from build123d import *

# Parameters (mm, degrees)
SKETCH_1_W              = 95
SKETCH_1_H              = 65
EXTRUDE_1_DEPTH         = 12
HOLE_WIZARD_6_5_6_5_1_D = 6.5
CHAMFER_1_SIZE          = 5
SKETCH_4_R              = 26
CUT_EXTRUDE_1_DEPTH     = 59.792006259
HOLE_WIZARD_M5_1_D      = 4.2
CHAMFER_2_SIZE          = 1


with BuildPart() as part:
    # 草图1 → 凸台-拉伸1 (new body)
    with BuildSketch(Plane.XY):
        Rectangle(SKETCH_1_W, SKETCH_1_H)
    extrude(amount=EXTRUDE_1_DEPTH)

    # Ø6.5 (6.5) 直径孔1 (through all)
    with Locations(Plane.XY.offset(12)):
        with Locations((-40, -26.5), (40, -26.5)):
            Hole(HOLE_WIZARD_6_5_6_5_1_D / 2)

    # 倒角1
    chamfer_1_edges = [part.edges().sort_by_distance(p)[0] for p in [
        (-47.5, 32.5, 6),
        (47.5, 32.5, 6),
    ]]
    chamfer(chamfer_1_edges, length=CHAMFER_1_SIZE)

    # 草图4 → 切除-拉伸1 (cut, through all)
    with BuildSketch(Plane(origin=(0, 0, 0), x_dir=(-1, 0, 0), z_dir=(0, 0, -1))):
        with Locations((0, 2.5)):
            Circle(SKETCH_4_R)
    extrude(amount=-CUT_EXTRUDE_1_DEPTH, mode=Mode.SUBTRACT)

    # M5 螺纹孔1 (through all)
    with Locations(Plane.XY.offset(12)):
        with Locations((-24.748737342, 27.25), (24.748737342, 27.25), (24.748737342, -22.25), (-24.748737342, -22.25)):
            Hole(HOLE_WIZARD_M5_1_D / 2)

    # 倒角2
    chamfer_2_edges = [part.edges().sort_by_distance(p)[0] for p in [
        (0, -32.5, 12),
        (0, 32.5, 0),
        (0, 32.5, 12),
        (-47.5, -2.5, 0),
        (-45, 30, 0),
        (45, 30, 0),
        (-47.5, -2.5, 12),
        (-45, 30, 12),
        (45, 30, 12),
        (47.5, -2.5, 12),
        (0, -32.5, 0),
        (47.5, -2.5, 0),
        (47.5, -32.5, 6),
        (-47.5, -32.5, 6),
    ]]
    chamfer(chamfer_2_edges, length=CHAMFER_2_SIZE)


solid = part.part
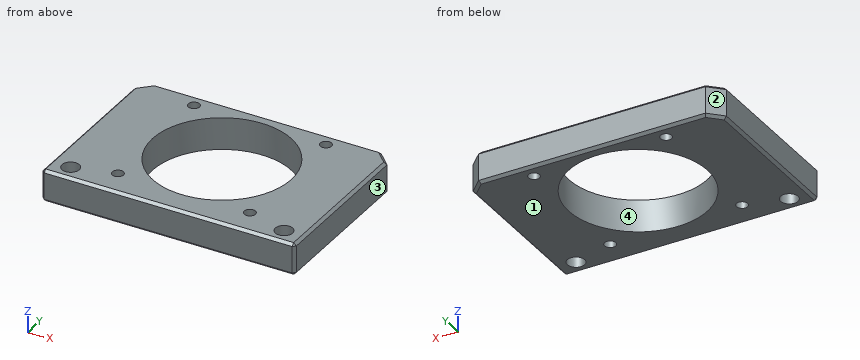
Could you check a few things on this model? Use its own coordinates, in mm. Face numbers are marked on the shaded views. Coordinates: 2 decimals unless noted, no trailing zeros. Order: outer loops, then holes, each group sorted by start corner. A loop starts at its lowest first (then second) coordinate and runs counter-clockwise, first axis right, second up.
Q1. Thinking about a two-plate mould opening in X: for the marked faces 1, 2, 3 and 4, which applies, released by +X, released by -X, zero draft, split by the parting line, or undercut?
Q2. Suppose I cut it at D-D on z = 3. Please give me the cut outline in (x, y), and give its area (3 significant figures).
Q3. Suppose I cut it at C-C on y = 2.5. Please give me the cut outline in (x, z), and give its area (3 significant figures).
Q4. Please list where these lines run through material, in increasing order: L1, parallel to Y at x = 40, z = 5; L2, parallel to X at y = 26.5, z = 2; L3, parallel to Y at x = -4, z = 3.25.
Q5. Suppose I cut it at A-A on x = -40. Please give me the cut outline in (y, z).
Q6. Suppose I cut it at B-B on y = -26.5. Please give me the cut outline in (x, z), and give its area (3 significant figures).
Answer:
1. face 1: zero draft
1. face 2: released by -X
1. face 3: released by +X
1. face 4: undercut
2. outline: (-47.5, -31.5) - (-46.5, -32.5) - (46.5, -32.5) - (47.5, -31.5) - (47.5, 27.5) - (42.5, 32.5) - (-42.5, 32.5) - (-47.5, 27.5) - close; hole circle Ø6.5 at (-40, -26.5); hole circle Ø4.2 at (-24.75, -22.25); hole circle Ø4.2 at (-24.75, 27.25); hole circle Ø52 at (0, 2.5); hole circle Ø4.2 at (24.75, -22.25); hole circle Ø4.2 at (24.75, 27.25); hole circle Ø6.5 at (40, -26.5)
2. area: 3,900 mm2
3. outline: (-47.5, 1) - (-46.5, 0) - (-26, 0) - (-26, 12) - (-46.5, 12) - (-47.5, 11) - close; (26, 0) - (46.5, 0) - (47.5, 1) - (47.5, 11) - (46.5, 12) - (26, 12) - close
3. area: 514 mm2
4. L1: y = -32.5 to -29.75, -23.25 to 32.5
4. L2: x = -47.5 to -26.71, -22.79 to -10, 10 to 22.79, 26.71 to 47.5
4. L3: y = -32.5 to -23.19, 28.19 to 32.5
5. outline: (-32.5, 1) - (-31.5, 0) - (-29.75, 0) - (-29.75, 12) - (-31.5, 12) - (-32.5, 11) - close; (-23.25, 0) - (31.5, 0) - (32.5, 1) - (32.5, 11) - (31.5, 12) - (-23.25, 12) - close
6. outline: (-47.5, 1) - (-46.5, 0) - (-43.25, 0) - (-43.25, 12) - (-46.5, 12) - (-47.5, 11) - close; (-36.75, 0) - (36.75, 0) - (36.75, 12) - (-36.75, 12) - close; (43.25, 0) - (46.5, 0) - (47.5, 1) - (47.5, 11) - (46.5, 12) - (43.25, 12) - close
6. area: 982 mm2
